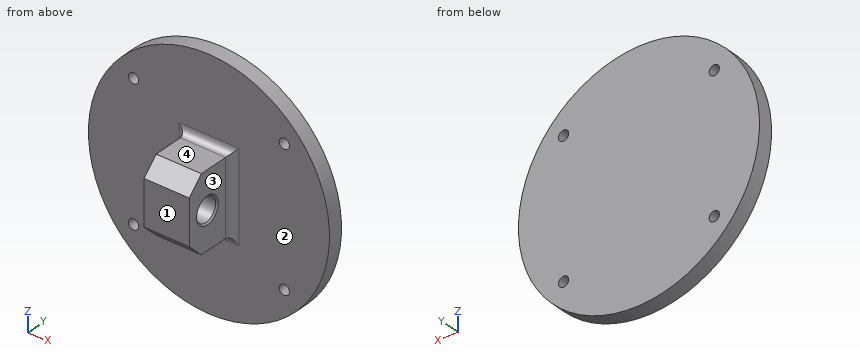
```python
from build123d import *

# Parameters (mm, degrees)
SKETCH1_R           = 80
BOSS_EXTRUDE1_DEPTH = 5
M8_TAPPED_HOLE1_D   = 6.8
SKETCH7_W           = 30
SKETCH7_H           = 50
BOSS_EXTRUDE2_DEPTH = 35
SKETCH8_R           = 8
CUT_EXTRUDE4_DEPTH  = 131.479883507
CHAMFER1_SIZE       = 10
FILLET3_R           = 5
CHAMFER2_SIZE       = 1


with BuildPart() as part:
    # Sketch1 → Boss-Extrude1 (new, symmetric)
    with BuildSketch(Plane(origin=(0, 0, 0), x_dir=(1, 0, 0), z_dir=(0, 1, 0))):
        with Locations(Location((0, 0, 0), (0, 0, 270))):
            Circle(SKETCH1_R)
    extrude(amount=BOSS_EXTRUDE1_DEPTH, both=True)

    # M8 Tapped Hole1 (through all)
    with Locations(Plane(origin=(0, -5, 0), x_dir=(-1, 0, 0), z_dir=(0, -1, 0))):
        with Locations((50, -45), (50, 45), (-50, 45), (-50, -45)):
            Hole(M8_TAPPED_HOLE1_D / 2)

    # Sketch7 → Boss-Extrude2 (add)
    with BuildSketch(Plane.XZ.offset(5)):
        Rectangle(SKETCH7_W, SKETCH7_H)
    extrude(amount=BOSS_EXTRUDE2_DEPTH)

    # Sketch8 → Cut-Extrude4 (cut, through all)
    with BuildSketch(Plane(origin=(15, 0, 0), x_dir=(0, 0, -1), z_dir=(1, 0, 0))):
        with Locations((0, -25)):
            Circle(SKETCH8_R)
    extrude(amount=-CUT_EXTRUDE4_DEPTH, mode=Mode.SUBTRACT)

    # Chamfer1
    chamfer1_edges = [part.edges().sort_by_distance(p)[0] for p in [
        (0, -40, 25),
        (0, -40, -25),
    ]]
    chamfer(chamfer1_edges, length=CHAMFER1_SIZE)

    # Fillet3
    fillet3_edges = [part.edges().sort_by_distance(p)[0] for p in [
        (15, -5, 0),
        (0, -5, 25),
        (-15, -5, 0),
        (0, -5, -25),
    ]]
    fillet(fillet3_edges, radius=FILLET3_R)

    # Chamfer2
    chamfer2_edges = [part.edges().sort_by_distance(p)[0] for p in [
        (-15, -25, 8),
        (15, -25, 8),
    ]]
    chamfer(chamfer2_edges, length=CHAMFER2_SIZE)


solid = part.part
```
Work out the finished part from the listing and answer in its coordinate system (mm). Face numbers are marked on the shaded views. A direction names the side the tool comes from. Give positions to 0.01 mm unless a question says otherwise; leave off trailing zeros. Order: outer loops, then holes, each group sorted by start corner. A loop starts at its lowest first (then second) coordinate and runs counter-clockwise, first axis right, second up. Notation, with made-up numbers: M -28.75,56 L -19.75,56 A9 cw -19.75,65 Z; hole C 18,-24 d2. An arc over 180 degrees is marked long. Return JSON: item names as keys, results as strings.
1) Straight lines are drawn through the part: line 1 along Z through (x, y) = (50, 0); line 2 along Y through (x, z) = (-2.25, 0); line 3 along X through (y, z) = (1, 45). For each, find the intervals that lie inside material, in ascending order. Write a range as [from, to].
Resolved:
{"line 1": "[-62.45, -48.4], [-41.6, 41.6], [48.4, 62.45]", "line 2": "[-40, -33], [-17, 5]", "line 3": "[-66.14, -53.4], [-46.6, 46.6], [53.4, 66.14]"}
2) Section D-D, the plane z = -45 is taken. Write down the section's boundary in (x, y), plus the area to 3 significant figures.
Resolved:
{"outline": "M -66.14,-5 L -53.4,-5 L -53.4,5 L -66.14,5 Z; M -46.6,-5 L 46.6,-5 L 46.6,5 L -46.6,5 Z; M 53.4,-5 L 66.14,-5 L 66.14,5 L 53.4,5 Z", "area": "1,190 mm^2"}
3) Section A-A, the plane z = 0 is taken. Write down the section's boundary in (x, y).
Resolved:
{"outline": "M -80,-5 L -20,-5 A5 cw -15,-10 L -15,-16 L -14,-17 L 14,-17 L 15,-16 L 15,-10 A5 cw 20,-5 L 80,-5 L 80,5 L -80,5 Z; M -15,-40 L 15,-40 L 15,-34 L 14,-33 L -14,-33 L -15,-34 Z"}
4) Section B-B, the plane y = -25 is taken. Write down the section's boundary in (x, z).
Resolved:
{"outline": "M -15,-25 L 15,-25 L 15,-9 L 14,-8 L -14,-8 L -15,-9 Z; M -15,9 L -14,8 L 14,8 L 15,9 L 15,25 L -15,25 Z"}
5) Each of these flat-tipped pins is pushed along its axis until it touches: pin 1 (1 mm diameter, centred on x = 21, z = 27.5, fed in from -Y); pin 2 (10 mm diameter, centred on y = -6.5, z = 47.5, fed in from +X); pin 3 (6 mm diameter, centred on x = -6.5, y = -21.5, fed in from -Z); pin 4 (14.5 mm diameter, centred on y = -25, z = 0, fed in from +X). Where does it stop, or does it pass through?
Resolved:
{"pin 1": "y = -5", "pin 2": "x = 67.63", "pin 3": "z = -25", "pin 4": "through"}
6) A tool of negligible diameter and unlimited length cuts with its end or side. For the marked faces 1, 2, 3 and 4, from which of +Z, -Z, +X, -X, +Y, -Y can it reach the whole face along a straight path? Write none if from no direction.
Resolved:
{"face 1": "+Z, -Z, +X, -X, -Y", "face 2": "-Y", "face 3": "+Z, -Z, +X, -Y", "face 4": "+Z, +X, -X, -Y"}
7) Section C-C, the plane x = 0 is taken. Write down the section's boundary in (y, z), plus the area to 3 significant figures.
Resolved:
{"outline": "M -40,-15 L -30,-25 L -10,-25 A5 cw -5,-30 L -5,-80 L 5,-80 L 5,80 L -5,80 L -5,30 A5 cw -10,25 L -30,25 L -40,15 Z; hole C -25,0 d16", "area": "3,060 mm^2"}
